Can you work these out from the model? Positions are in its coordinate system, mm. Round coordinates to 2 decimals unless told otherwise and drop trailing zeros. Loops run counter-clockwise (first coordinate to the right, second up) from the corner with the lowest first, then second, coordinate; pieces in that order, holes last.
from build123d import *

# Parameters (mm, degrees)
SKETCH_1_W         = 76
SKETCH_1_H         = 41.5
EXTRUDE_1_DEPTH    = 65
HOLE_WIZARD_M6_1_D = 5
CHAMFER_1_SIZE     = 2


with BuildPart() as part:
    # 草图1 → 凸台-拉伸1 (new, symmetric)
    with BuildSketch(Plane.XY):
        Rectangle(SKETCH_1_W, SKETCH_1_H)
    extrude(amount=EXTRUDE_1_DEPTH, both=True)

    # M6 螺纹孔1 (through all)
    with Locations(Plane(origin=(0, 20.75, 0), x_dir=(1, 0, 0), z_dir=(0, 1, 0))):
        with Locations((-27.000001035, -50), (27.000001035, -50), (27.000001035, 50), (-27.000001035, 50)):
            Hole(HOLE_WIZARD_M6_1_D / 2)

    # 倒角1
    chamfer_1_edges = [part.edges().sort_by_distance(p)[0] for p in [
        (-38, 0, 65),
        (38, 0, 65),
        (-38, 0, -65),
        (38, 0, -65),
    ]]
    chamfer(chamfer_1_edges, length=CHAMFER_1_SIZE)


solid = part.part
(1) If we section it at A-A, the plane z = 50: List the corners of the cut face in (x, y) for me, then the cut area to 3 significant figures.
Worked answers:
outline: (-38, -20.75) - (-29.5, -20.75) - (-29.5, 20.75) - (-38, 20.75) - close; (-24.5, -20.75) - (24.5, -20.75) - (24.5, 20.75) - (-24.5, 20.75) - close; (29.5, -20.75) - (38, -20.75) - (38, 20.75) - (29.5, 20.75) - close
area: 2,740 mm2
(2) Will this pin go through, and if not, where does the flat tip stop? P1, Ø4.5, axis at x = -27, z = 50, coming from the -Y side.
Worked answers:
P1: passes through
(3) If I drill on line 1 (X direction, y = -4.5, z = -50), over which ranges is the centre line in solid material (lowest first)?
Worked answers:
line 1: x = -38 to -29.5, -24.5 to 24.5, 29.5 to 38
(4) If we mould it in two halves opening along Z, with no side actions, what happens to faces 1 (the flat face through (-1, 0, -65)), 2 (the flat face through (-1, -20.75, 1)), 3 (the cylindrical face through (-26.46, -0.29, 52.44))? For each: released by +Z, released by -Z, zero draft, split by the parting line, or undercut.
Worked answers:
face 1: released by -Z
face 2: zero draft
face 3: undercut
